CAD build for the part. Positions are in the model's coordinates, mm. Face numbers are marked on the shaded views. A direction names the side the tool comes from. Give positions to 0.01 mm unless a question says otherwise; leave off trailing zeros. Write each loop counter-clockwise with the first axis right and the second up, starting at its lowest first coordinate (ties: lowest second). Pieces come first, ordered by that corner, then holes. Notation, with made-up numbers: (30, -32.75) -> (89, -32.75) arc R31 ccw to (89, -1.75) -> close; hole circle Ø2 at (-20.5, 64). An arc over 180 degrees is marked (long way). Answer in a Markdown table with one row per item. Add a question column.
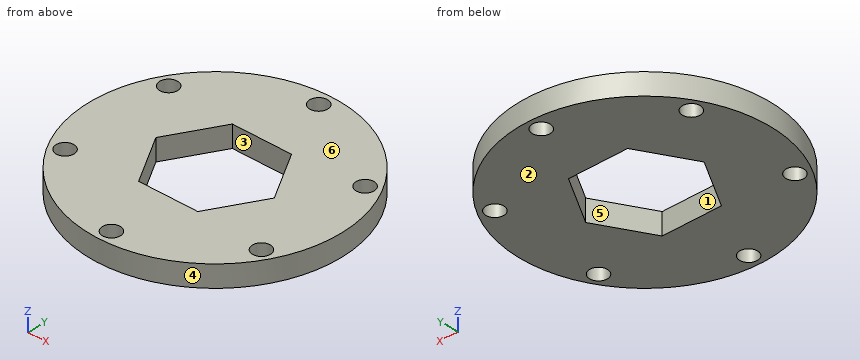
```python
from build123d import *

# Parameters (mm, degrees)
SKETCH1_R           = 70
SKETCH1_R_2         = 5
BOSS_EXTRUDE1_DEPTH = 12


with BuildPart() as part:
    # Sketch1 → Boss-Extrude1 (new body)
    with BuildSketch(Plane.XY):
        Circle(SKETCH1_R)
        with Locations((0, 62.5)):
            Circle(SKETCH1_R_2, mode=Mode.SUBTRACT)
        with Locations((54.126587737, 31.25)):
            Circle(SKETCH1_R_2, mode=Mode.SUBTRACT)
        with Locations((54.126587737, -31.25)):
            Circle(SKETCH1_R_2, mode=Mode.SUBTRACT)
        with Locations((0, -62.5)):
            Circle(SKETCH1_R_2, mode=Mode.SUBTRACT)
        with Locations((-54.126587737, -31.25)):
            Circle(SKETCH1_R_2, mode=Mode.SUBTRACT)
        with Locations((-54.126587737, 31.25)):
            Circle(SKETCH1_R_2, mode=Mode.SUBTRACT)
        Polygon((32.620290209, 0), (16.310145105, 28.25), (-16.310145105, 28.25), (-32.620290209, 0), (-16.310145105, -28.25), (16.310145105, -28.25), align=None, mode=Mode.SUBTRACT)
    extrude(amount=BOSS_EXTRUDE1_DEPTH)


solid = part.part
```
Item 1: Probe L1, parallel to Y at x = 0, z = 5.5; L2, parallel to X at y = 27, z = 5.75; L3, parallel to Y at x = 1, z = 8.5. List the from-to ranges inside material, lowest first. Write a range as from..to.
Item 2: Which spindle directions (+Z, -Z, +X, -X, +Y, -Y) get a long thin tool onto all of the face, cutting with end or side? Do the marked faces 1 and 2. Say none if no direction does.
Item 3: Mould opens along X. For the marked faces 3, 4, 5 and 6 say: released by +X, released by -X, zero draft, split by the parting line, or undercut.
Item 4: Slice it at A-A, the plane x = 0. List the corners of the cut face in (y, z).
Item 5: Slice it at D-D, the plane x = 31. List the corners of the cut face in (y, z), then the cut area to 3 significant figures.
Item 6: Drop flat-ended pins along their axis: pin 1 Ø3.5 at (x, z) = (-8, 8) entering from -Y; pin 2 Ø1 at (x, z) = (-21, 1) entering from -Y; pin 3 Ø11.5 at (x, y) = (0, -62.5) entering from -Z; pin 4 Ø3 at (y, z) = (28, 6) entering from -X. Give the stop position or say it passes through.
Item 7: Slice it at C-C, the plane x = -51. List the corners of the cut face in (y, z), then the cut area to 3 significant figures.
Item 8: Slice it at B-B, the plane y = 62.5. List the corners of the cut face in (x, z).
Answer key:
| question | item | result |
|---|---|---|
| 1 | L1 | y = -70..-67.5, -57.5..-28.25, 28.25..57.5, 67.5..70 |
| 1 | L2 | x = -64.58..-56.76, -51.49..-17.03, 17.03..51.49, 56.76..64.58 |
| 1 | L3 | y = -69.99..-67.4, -57.6..-28.25, 28.25..57.6, 67.4..69.99 |
| 2 | face 1 | +Z, -Z |
| 2 | face 2 | -Z, +X, -X, +Y, -Y |
| 3 | face 3 | undercut |
| 3 | face 4 | split by the parting line |
| 3 | face 5 | undercut |
| 3 | face 6 | zero draft |
| 4 | outline | (-70, 0) -> (-67.5, 0) -> (-67.5, 12) -> (-70, 12) -> close; (-57.5, 0) -> (-28.25, 0) -> (-28.25, 12) -> (-57.5, 12) -> close; (28.25, 0) -> (57.5, 0) -> (57.5, 12) -> (28.25, 12) -> close; (67.5, 0) -> (70, 0) -> (70, 12) -> (67.5, 12) -> close |
| 5 | outline | (-62.76, 0) -> (-2.81, 0) -> (-2.81, 12) -> (-62.76, 12) -> close; (2.81, 0) -> (62.76, 0) -> (62.76, 12) -> (2.81, 12) -> close |
| 5 | area | 1,440 mm² |
| 6 | pin 1 | stops at y = -69.72 |
| 6 | pin 2 | stops at y = -66.93 |
| 6 | pin 3 | stops at z = 0 |
| 6 | pin 4 | stops at x = -64.79 |
| 7 | outline | (-47.95, 0) -> (-35.15, 0) -> (-35.15, 12) -> (-47.95, 12) -> close; (-27.35, 0) -> (27.35, 0) -> (27.35, 12) -> (-27.35, 12) -> close; (35.15, 0) -> (47.95, 0) -> (47.95, 12) -> (35.15, 12) -> close |
| 7 | area | 963 mm² |
| 8 | outline | (-31.52, 0) -> (-5, 0) -> (-5, 12) -> (-31.52, 12) -> close; (5, 0) -> (31.52, 0) -> (31.52, 12) -> (5, 12) -> close |
